```python
from build123d import *

# Parameters (mm, degrees)
BASE_EXTRUDE_DEPTH = 22
FILLET1_R          = 1.2


with BuildPart() as part:
    # Sketch1 → Base-Extrude (new body)
    with BuildSketch(Plane.XY):
        with BuildLine():
            Line((-80, 20), (80, 20))
            ThreePointArc((80, 20), (100, 0), (80, -20))
            Line((80, -20), (-80, -20))
            ThreePointArc((-80, -20), (-100, 0), (-80, 20))
        make_face()
    extrude(amount=BASE_EXTRUDE_DEPTH)

    # Fillet1
    fillet1_edges = [part.edges().sort_by_distance(p)[0] for p in [
        (100, 0, 22),
        (0, 20, 22),
        (-100, 0, 22),
        (0, 20, 0),
        (100, 0, 0),
        (0, -20, 0),
        (-100, 0, 0),
        (0, -20, 22),
    ]]
    fillet(fillet1_edges, radius=FILLET1_R)


solid = part.part
```
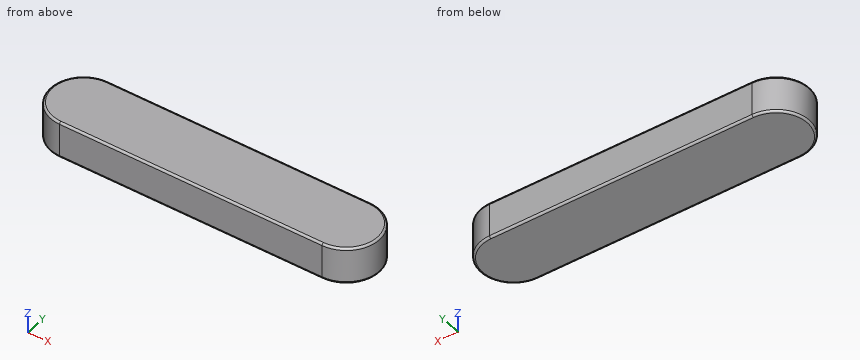
CAD build for the part. Positions are in the model's coordinates, mm. Coordinates: 2 decimals unless noted, no trailing zeros. Order: outer loops, then holes, each group sorted by start corner. A loop starts at its lowest first (then second) coordinate and runs counter-clockwise, first axis right, second up.
(1) Pin check, flat tips, straight feed: pin 1 Ø10 at (y, z) = (-4, 17.5) entering from -X; pin 2 Ø4 at (y, z) = (9.5, 16) entering from +X; pin 3 Ø12 at (y, z) = (8.5, 16) entering from +X. Stop position of each tip, or through.
Solution:
pin 1: stops at x = -100
pin 2: stops at x = 98.54
pin 3: stops at x = 99.84
(2) Drill centre lines: L1, parallel to X at y = -4, z = 2; L2, parallel to X at y = -7.5, z = 19.5; L3, parallel to Y at x = 91, z = 18. Where is each one in solid material? Low to high.
Solution:
L1: x = -99.6 to 99.6
L2: x = -98.54 to 98.54
L3: y = -16.7 to 16.7
(3) Saw through at A-A, the plane z = 6. Write the cut outline in (x, y).
Solution:
outline: (-80, -20) - (80, -20) arc R20 ccw to (80, 20) - (-80, 20) arc R20 ccw to start
